from build123d import *

# Parameters (mm, degrees)
SKETCH_1_W          = 80
SKETCH_1_H          = 90
SKETCH_1_W_2        = 130
EXTRUDE_1_DEPTH     = 3
SKETCH_2_W          = 3
SKETCH_2_H          = 90
EXTRUDE_2_DEPTH     = 25
SKETCH_3_R          = 10
SKETCH_3_R_2        = 3
CUT_EXTRUDE_1_DEPTH = 25


with BuildPart() as part:
    # 草图1 → 凸台-拉伸1 (new body)
    with BuildSketch(Plane.XY):
        with Locations((-65, 135)):
            Rectangle(SKETCH_1_W, SKETCH_1_H)
        with Locations((-65, 45)):
            Rectangle(SKETCH_1_W_2, SKETCH_1_H)
    extrude(amount=EXTRUDE_1_DEPTH)

    # 草图2 → 凸台-拉伸2 (add)
    with BuildSketch(Plane.XY.offset(3)):
        with Locations((-103.5, 135)):
            Rectangle(SKETCH_2_W, SKETCH_2_H)
        with Locations((-26.5, 135)):
            Rectangle(SKETCH_2_W, SKETCH_2_H)
    extrude(amount=EXTRUDE_2_DEPTH)

    # 草图3 → 切除-拉伸1 (cut)
    with BuildSketch(Plane(origin=(0, 0, 0), x_dir=(-1, 0, 0), z_dir=(0, 0, -1))):
        with Locations((65, 45)):
            Circle(SKETCH_3_R)
        with Locations((12.5, 15)):
            Circle(SKETCH_3_R_2)
        with Locations((65, 15)):
            Circle(SKETCH_3_R_2)
        with Locations((117.5, 15)):
            Circle(SKETCH_3_R_2)
        with Locations((117.5, 75)):
            Circle(SKETCH_3_R_2)
        with Locations((65, 75)):
            Circle(SKETCH_3_R_2)
        with Locations((12.5, 75)):
            Circle(SKETCH_3_R_2)
    extrude(amount=-CUT_EXTRUDE_1_DEPTH, mode=Mode.SUBTRACT)


solid = part.part
Source: CAD feature listing. Evaluate the final solid. Frame: model axes, mm. A direction names the side the tool comes from. Coordinates: 2 decimals unless noted, no trailing zeros. Order: outer loops, then holes, each group sorted by start corner. A loop starts at its lowest first (then second) coordinate and runs counter-clockwise, first axis right, second up. Notation, with made-up numbers: M 53,37 L 79,37 A5 cw 79,46 Z; hole C 88,-36 d1. An arc over 180 degrees is marked long. Write each question's results on one line, items separated by ' | '. Start each with the question number.
1. Reachability of faces 1 (the face through (-62.6, 73.2, 1.5)), 2 (the face through (-28, 134, 15)) from +Z, -Z, +X, -X, +Y, -Y: full face, straight path, thin tool, end or side. Return the list, or none.
2. Pin query (flat end, axial travel): pin 1 (18 mm diameter, centred on x = -65, y = 45, fed in from +Z); pin 2 (9.5 mm diameter, centred on x = -117.5, y = 75, fed in from -Z); pin 3 (2 mm diameter, centred on x = -24.5, z = 20.5, fed in from -Y); pin 4 (12 mm diameter, centred on y = 88.5, z = 19.5, fed in from -X). Return the tip coordinate at first contact, or that it passes through.
3. Draft query along X for faces 3 (the face through (-102, 134, 15)), 4 (the face through (-66, 71, 0)), 5 (the face through (-25, 134, 14)). Return one class per face: +X half, -X half, draft (parallel to the pull), parting line (faces both ways), or undercut.
4. Section A-A, the plane x = -65. Return the cut outline in (y, z), then the cut area to 3 significant figures.
5. Section D-D, the plane z = 19.25. Return the cut outline in (x, y), then the cut area to 3 significant figures.
6. Section C-C, the plane x = -12.5. Return the cut outline in (y, z).
7. Section B-B, the plane y = 75. Return the cut outline in (x, z).
8. Material intervals for L1, parallel to Y at x = -117.5, z = 1.4; L2, parallel to Y at x = -65, z = 1.95; L3, parallel to X at y = 107, z = 14, sorted ascending.
Solution:
1) face 1: +Z, -Z | face 2: +Z, +Y, -Y
2) pin 1: through | pin 2: z = 0 | pin 3: y = 90 | pin 4: x = -105
3) face 3: undercut | face 4: draft | face 5: +X half
4) outline: M 0,0 L 12,0 L 12,3 L 0,3 Z; M 18,0 L 35,0 L 35,3 L 18,3 Z; M 55,0 L 72,0 L 72,3 L 55,3 Z; M 78,0 L 180,0 L 180,3 L 78,3 Z | area: 444 mm²
5) outline: M -105,90 L -102,90 L -102,180 L -105,180 Z; M -28,90 L -25,90 L -25,180 L -28,180 Z | area: 540 mm²
6) outline: M 0,0 L 12,0 L 12,3 L 0,3 Z; M 18,0 L 72,0 L 72,3 L 18,3 Z; M 78,0 L 90,0 L 90,3 L 78,3 Z
7) outline: M -130,0 L -120.5,0 L -120.5,3 L -130,3 Z; M -114.5,0 L -68,0 L -68,3 L -114.5,3 Z; M -62,0 L -15.5,0 L -15.5,3 L -62,3 Z; M -9.5,0 L 0,0 L 0,3 L -9.5,3 Z
8) L1: 0 to 12, 18 to 72, 78 to 90 | L2: 0 to 12, 18 to 35, 55 to 72, 78 to 180 | L3: -105 to -102, -28 to -25
